Input: part model. Units: mm. Frame: model coordinates. A direction names the side the tool comes from. Coordinates: 2 decimals unless noted, no trailing zeros. Order: outer loops, then holes, each group sorted by start corner. A loop starts at its lowest first (then second) coordinate and runs counter-clockwise, first axis right, second up. Notation, with made-up numbers: (6.25, 79.5) - (50.25, 79.5) arc R22 cw to (50.25, 98.5) - close; hole circle Ø5 at (43.25, 27.5). An arc over 180 degrees is marked (long way). One line per question, with ' | ' between items. Start each with the question number.
```python
from build123d import *

# Parameters (mm, degrees)
EXTRUDE_263_DEPTH   = 120
EXTRUDE_1_DEPTH     = 6
EXTRUDE_START       = 6
EXTRUDE_2_DEPTH     = 6
SKETCH_4_R          = 2.5
CUT_EXTRUDE_1_DEPTH = 10
SKETCH_5_W          = 16
SKETCH_5_H          = 120
CUT_EXTRUDE_2_DEPTH = 0.65


with BuildPart() as part:
    # 草图1 → Extrude 263 (new body)
    with BuildSketch(Plane.XY):
        with BuildLine():
            Line((0, 0), (40, 0))
            Line((40, 0), (40, 8))
            ThreePointArc((40, 8), (39.121320344, 10.121320344), (37, 11))
            Line((37, 11), (3, 11))
            ThreePointArc((3, 11), (0.878679656, 10.121320344), (0, 8))
            Line((0, 8), (0, 0))
        make_face()
    extrude(amount=-EXTRUDE_263_DEPTH)

    # 草图2 → 凸台-拉伸1 (add)
    with BuildSketch(Plane.XY):
        with BuildLine():
            Line((1, 0), (39, 0))
            Line((39, 0), (39, 6.5))
            ThreePointArc((39, 6.5), (38.121320344, 8.621320344), (36, 9.5))
            Line((36, 9.5), (4, 9.5))
            ThreePointArc((4, 9.5), (1.878679656, 8.621320344), (1, 6.5))
            Line((1, 6.5), (1, 0))
        make_face()
    extrude(amount=EXTRUDE_1_DEPTH)

    # 草图3 → 凸台-拉伸2 (add)
    with BuildSketch(Plane(origin=(0, 0, -120), x_dir=(-1, 0, 0), z_dir=(0, 0, -1)).offset(EXTRUDE_START)):
        with BuildLine():
            Line((-39, 0), (-1, 0))
            Line((-1, 0), (-1, 6.5))
            ThreePointArc((-1, 6.5), (-1.878679656, 8.621320344), (-4, 9.5))
            Line((-4, 9.5), (-36, 9.5))
            ThreePointArc((-36, 9.5), (-38.121320344, 8.621320344), (-39, 6.5))
            Line((-39, 6.5), (-39, 0))
        make_face()
    extrude(amount=-EXTRUDE_2_DEPTH)

    # 草图4 → 切除-拉伸1 (cut)
    with BuildSketch(Plane(origin=(0, 11, 0), x_dir=(-1, 0, 0), z_dir=(0, 1, 0))):
        with Locations(Location((-33, -10, 0), (0, 0, 90))):
            Circle(SKETCH_4_R)
        with Locations(Location((-7, -10, 0), (0, 0, 90))):
            Circle(SKETCH_4_R)
        with Locations(Location((-33, -33, 0), (0, 0, 90))):
            Circle(SKETCH_4_R)
        with Locations(Location((-7, -33, 0), (0, 0, 90))):
            Circle(SKETCH_4_R)
        with Locations(Location((-7, -87, 0), (0, 0, 270))):
            Circle(SKETCH_4_R)
        with Locations(Location((-33, -87, 0), (0, 0, 270))):
            Circle(SKETCH_4_R)
        with Locations(Location((-7, -110, 0), (0, 0, 270))):
            Circle(SKETCH_4_R)
        with Locations(Location((-33, -110, 0), (0, 0, 270))):
            Circle(SKETCH_4_R)
    extrude(amount=-CUT_EXTRUDE_1_DEPTH, mode=Mode.SUBTRACT)

    # 草图5 → 切除-拉伸2 (cut)
    with BuildSketch(Plane(origin=(0, 11, 0), x_dir=(-1, 0, 0), z_dir=(0, 1, 0))):
        with Locations((-20, -60)):
            Rectangle(SKETCH_5_W, SKETCH_5_H)
    extrude(amount=-CUT_EXTRUDE_2_DEPTH, mode=Mode.SUBTRACT)


solid = part.part
```
(1) Draft query along X for faces 6 (the face through (20, 10, 0)), 7 (the face through (38.1, 8.64, -123.04)), 8 (the face through (7, 1, -87)). Return one class per face: +X half, -X half, draft (parallel to the pull), parting line (faces both ways), or undercut.
(2) Section B-B (z = -97). Output: boundary loops of the cut face in (x, y), then the cut area to 3 significant figures.
(3) Section C-C (y = 2.5). State how many separate pieces and enclosed holes the cut face has, then the cut area to 3 significant figures.
(4) Material intervals for line 1 along X through (y, z) = (8.25, -10); line 2 along Z through (x, y) = (6, 2); line 3 along Y through (x, z) = (15, -69), sorted ascending. Write a range as from..to.
(5) Pin query (flat end, axial travel): pin 1 (1 mm diameter, centred on y = 9, z = -94, fed in from +X); pin 2 (4 mm diameter, centred on x = 33, z = -10, fed in from +Y); pin 3 (1.8 mm diameter, centred on x = 27, z = -123.5, fed in from +Y). Return the tip coordinate at first contact, or that it passes through.
(6) Section D-D (x = 17). Output: boundary loops of the cut face in (y, z).
(7) Reachability of faces 1 (the face through (1.9, 8.64, 2.96)), 2 (the face through (1, 3, -123)), 3 (the face through (1, 3, 3)), 4 (the face through (34.69, 6.07, -11.84)), 5 (the face through (1.86, 8.6, -123.04)) from +Z, -Z, +X, -X, +Y, -Y: full face, straight path, thin tool, end or side. Return the list, or none.
(8) Section A-A (x = 33). Output: boundary loops of the cut face in (y, z), then the cut area to 3 significant figures.
Worked answers:
1) face 6: draft | face 7: +X half | face 8: undercut
2) outline: (0, 0) - (40, 0) - (40, 8) arc R3 ccw to (37, 11) - (28, 11) - (28, 10.35) - (12, 10.35) - (12, 11) - (3, 11) arc R3 ccw to (0, 8) - close | area: 426 mm²
3) separate pieces: 1 | enclosed holes: 8 | area: 5,100 mm²
4) line 1: x = 0.01..4.5, 9.5..30.5, 35.5..39.99 | line 2: z = -126..-112.29, -107.71..-89.29, -84.71..-35.29, -30.71..-12.29, -7.71..6 | line 3: y = 0..10.35
5) pin 1: stops at x = 39.96 | pin 2: stops at y = 1 | pin 3: stops at y = 9.5
6) outline: (0, -126) - (9.5, -126) - (9.5, -120) - (10.35, -120) - (10.35, 0) - (9.5, 0) - (9.5, 6) - (0, 6) - close
7) face 1: +Z, -X, +Y | face 2: -Z, -X, +Y, -Y | face 3: +Z, -X, +Y, -Y | face 4: +Y | face 5: -Z, -X, +Y
8) outline: (0, -126) - (9.5, -126) - (9.5, -120) - (11, -120) - (11, -112.5) - (1, -112.5) - (1, -107.5) - (11, -107.5) - (11, -89.5) - (1, -89.5) - (1, -84.5) - (11, -84.5) - (11, -35.5) - (1, -35.5) - (1, -30.5) - (11, -30.5) - (11, -12.5) - (1, -12.5) - (1, -7.5) - (11, -7.5) - (11, 0) - (9.5, 0) - (9.5, 6) - (0, 6) - close | area: 1,230 mm²
